```python
from build123d import *

# Parameters (mm, degrees)
EXTRUDE_364_DEPTH      = 7.5
SKETCH_4_W             = 0.6
SKETCH_4_H             = 11.392304845
CHAMFER_2049_SIZE      = 1.4
FILLET_2094_R          = 0.6
PATTERN_LINEAR_1_COUNT = 10
PATTERN_LINEAR_1_PITCH = 1.666666667


with BuildPart() as part:
    # 草图1 → Extrude 364 (new body)
    with BuildSketch(Plane(origin=(0, 0, 0), x_dir=(0, 0, -1), z_dir=(1, 0, 0))):
        Polygon((9, 5.196152423), (9, -5.196152423), (0, -10.392304845), (-9, -5.196152423), (-9, 5.196152423), (0, 10.392304845), align=None)
    extrude(amount=EXTRUDE_364_DEPTH)

    # 草图2 → 凸台-旋转1 (revolve)
    with BuildSketch(Plane.XY, mode=Mode.PRIVATE) as revolve_1_sk:
        Polygon((0, 0), (42.5, 0), (42.5, 4.4845), (42.5, 6), (7.791693541, 6), (0, 6), align=None)
    revolve(revolve_1_sk.sketch.rotate(Axis((0, 0, 0), (1, 0, 0)), 90), axis=Axis((0, 0, 0), (1, 0, 0)))

    # 草图3 → 切除-旋转1 (revolve, cut)
    with BuildSketch(Plane.XY):
        Polygon((0, 9), (3.690598923, 15.392304845), (3.690598923, 20.392304845), (-10, 20.392304845), (-10, 9), align=None)
    revolve(axis=Axis((0, 0, 0), (1, 0, 0)), mode=Mode.SUBTRACT)

    # 草图5 → 切除-旋转2 (revolve, cut)
    with BuildSketch(Plane.XY):
        Polygon((7.5, 9), (3.809401077, 15.392304845), (3.809401077, 20.392304845), (13.809401077, 20.392304845), (13.809401077, 9), align=None)
    revolve(axis=Axis((0, 0, 0), (1, 0, 0)), mode=Mode.SUBTRACT)

    # 草图4 → 切除-旋转3 (revolve, cut)
    with BuildSketch(Plane.XY, mode=Mode.PRIVATE) as cut_revolve_3_sk:
        with Locations((7.2, 14.696152423)):
            Rectangle(SKETCH_4_W, SKETCH_4_H)
    revolve(cut_revolve_3_sk.sketch.rotate(Axis((0, 0, 0), (1, 0, 0)), 270), axis=Axis((0, 0, 0), (1, 0, 0)), mode=Mode.SUBTRACT)

    # Chamfer 2049
    chamfer_2049_edges = [part.edges().sort_by_distance(p)[0] for p in [
        (42.5, 0, -6),
    ]]
    chamfer(chamfer_2049_edges, length=CHAMFER_2049_SIZE)

    # Fillet 2094
    fillet_2094_edges = [part.edges().sort_by_distance(p)[0] for p in [
        (7.5, 0, -6),
    ]]
    fillet(fillet_2094_edges, radius=FILLET_2094_R)

    # 草图6 → 切除-旋转4 (revolve, cut)
    with BuildSketch(Plane.XY):
        Polygon((27.5, -4.4845), (26.625025667, -6), (26.625025667, -7.5), (28.374974333, -7.5), (28.374974333, -6), align=None)
    cut_revolve_4 = revolve(axis=Axis((-3.175, 0, 0), (1, 0, 0)), mode=Mode.SUBTRACT)

    # 阵列(线性)1: 切除-旋转4 ×10
    with Locations(*[(i * PATTERN_LINEAR_1_PITCH, 0, 0) for i in range(1, PATTERN_LINEAR_1_COUNT)]):
        add(cut_revolve_4, mode=Mode.SUBTRACT)


solid = part.part
```
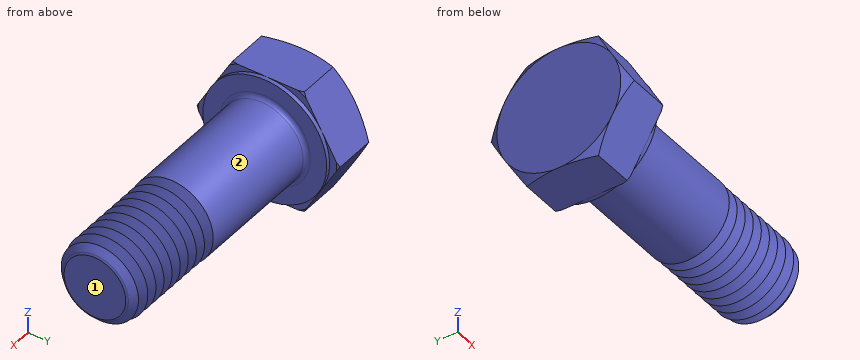
Geometry: final body of the model. Coordinates: model frame, mm. Face numbers are marked on the shaded views. A direction names the side the tool comes from. Coordinates: 2 decimals unless noted, no trailing zeros. Order: outer loops, then holes, each group sorted by start corner. A loop starts at its lowest first (then second) coordinate and runs counter-clockwise, first axis right, second up. Notation, with made-up numbers: (72.25, 35.5) - (87.25, 35.5) arc R30 ccw to (87.25, 64.5) - close; hole circle Ø10 at (28, 57.25). An arc over 180 degrees is marked (long way). Write each question's results on one line, items separated by ' | '.
(1) Line query: line 1 (X direction, y = -6.5, z = -5.25); line 2 (Y direction, x = 18, z = -1.75); line 3 (Z direction, x = 4, y = 6.5). Output: solid intervals per line, ascending. Write a range as [from, to].
Values found:
line 1: x = [0, 7.5] | line 2: y = [-5.74, 5.74] | line 3: z = [-6.74, 6.74]
(2) First-contact query: pin 1 Ø1 at (x, z) = (21, -4.5) entering from -Y; pin 2 Ø1.5 at (y, z) = (-8, 3.5) entering from +X; pin 3 Ø8 at (x, z) = (16.5, 3) entering from -Y. Flat tips, straight axial feed; report the tip coordinate or a pass-through.
Values found:
pin 1: stops at y = -4.47 | pin 2: stops at x = 7.5 | pin 3: stops at y = -6
(3) Set-up query: the marked faces 1 and 2. Return all of +Z, -Z, +X, -X, +Y, -Y with unobstructed straight access to the full face (end or side cutting, diameter ignored); none if empty.
Values found:
face 1: +Z, -Z, +X, +Y, -Y | face 2: +X
(4) Section query B-B, the plane x = 25.5. Return the cut outline in (y, z), plus the area to 3 significant figures.
Values found:
outline: circle Ø12 at (0, 0) | area: 113 mm²
(5) Section query A-A, the plane x = 4.5. Return the cut outline in (y, z), plus the area to 3 significant figures.
Values found:
outline: (-10.39, 0) - (-5.2, -9) - (5.2, -9) - (10.39, 0) - (5.2, 9) - (-5.2, 9) - close | area: 281 mm²
